Verification items for the finished model (mm, model axes). Face numbers are marked on the shaded views. Coordinates: 2 decimals unless noted, no trailing zeros. Write each loop counter-clockwise with the first axis right and the second up, starting at its lowest first coordinate (ties: lowest second). Pieces come first, ordered by that corner, then holes. Notation, with made-up numbers: (-7.5, 5.5) - (37.5, 5.5) arc R20 cw to (37.5, 10.5) - close; hole circle Ø2 at (-14.75, 86.5). An arc over 180 degrees is marked (long way). Use one line per item in the form item = value. Start each with the question number.
(1) Sectioned sample at C-C (x = 6.5). Record the cut outline in (y, z), and give its area (3 significant figures).
(2) Sectioned sample at B-B (y = -48). Record the cut outline in (x, z), and give its area (3 significant figures).
(3) Gauge pin test, flat ends, axial feed: pin 1 Ø4 at (y, z) = (24, -41.57) entering from -X; pin 2 Ø3 at (x, y) = (1.5, 21) entering from -Z; pin 3 Ø3 at (x, z) = (6, -33) entering from +Y; pin 4 Ø3 at (x, z) = (3, -19) entering from -Y. Record the tip position at first contact, or that the pin passes through.
(4) Sectioned sample at A-A (z = 0). Count the separate pieces of the cut face and the enclosed holes in it, and give its area (3 significant figures).
(5) Material ranges on line 1 (Y direction, x = 1.1, z = 0); line 2 (Y direction, x = 6.85, z = 0); line 3 (Z direction, x = 7, y = -15.5), recorded low to high. Write a range as [from, to].
(6) Mould release check, pull along Z, two halves, no side actions. Record for the marked faces 1, 2 and 3: released by +Z, released by -Z, zero draft, split by the parting line, or undercut.
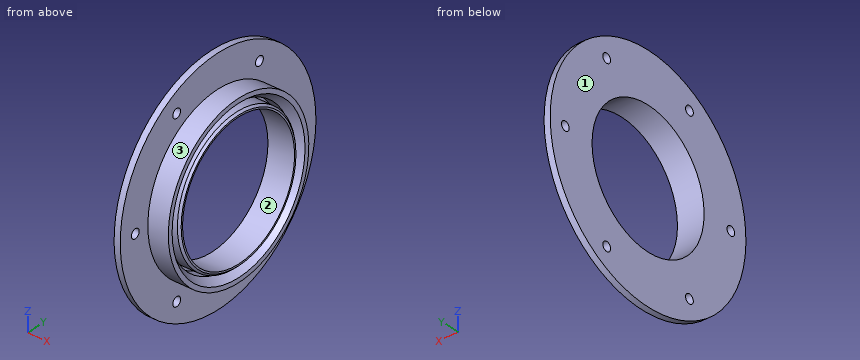
from build123d import *

# Parameters (mm, degrees)
CHAMFER1_SIZE      = 4
CHAMFER1_SIZE2     = 2.800830153
CHAMFER2_SIZE      = 1
SKETCH2_R          = 2.25
CUT_EXTRUDE1_DEPTH = 10
CIRPATTERN1_COUNT  = 6


with BuildPart() as part:
    # Sketch1 → Revolve1 (revolve)
    with BuildSketch(Plane.XY, mode=Mode.PRIVATE) as revolve1_sk:
        Polygon((0, 32.5), (13, 32.5), (13, 34.3), (3, 34.3), (3, 35.75), (13, 35.75), (13, 40.75), (3, 40.75), (3, 56.75), (0, 56.75), align=None)
    revolve(revolve1_sk.sketch.rotate(Axis((0, 0, 0), (1, 0, 0)), 90), axis=Axis((0, 0, 0), (1, 0, 0)))

    # Chamfer1
    chamfer1_edges = [part.edges().sort_by_distance(p)[0] for p in [
        (13, 0, -35.75),
    ]]
    chamfer1_side = [part.faces().sort_by_distance(p)[0] for p in [
        (8, 0, -35.75),
    ]]
    chamfer(chamfer1_edges, length=CHAMFER1_SIZE, length2=CHAMFER1_SIZE2, reference=chamfer1_side[0])

    # Chamfer2
    chamfer2_edges = [part.edges().sort_by_distance(p)[0] for p in [
        (13, 0, -34.3),
    ]]
    chamfer(chamfer2_edges, length=CHAMFER2_SIZE)

    # Sketch2 → Cut-Extrude1 (cut)
    with BuildSketch(Plane(origin=(3, 0, 0), x_dir=(0, 0, -1), z_dir=(1, 0, 0))):
        with Locations((0, 48)):
            Circle(SKETCH2_R)
    cut_extrude1 = extrude(amount=-CUT_EXTRUDE1_DEPTH, mode=Mode.SUBTRACT)

    # CirPattern1: Cut-Extrude1 ×6 about axis
    cirpattern1_axis = Axis((0, 0, 0), (1, 0, 0))
    for i in range(1, CIRPATTERN1_COUNT):
        add(cut_extrude1.rotate(cirpattern1_axis, i * 360 / CIRPATTERN1_COUNT), mode=Mode.SUBTRACT)


solid = part.part
Answers below:
q1.outline = circle Ø81.5 at (0, 0); circle Ø68.6 at (0, 0); hole circle Ø71.5 at (0, 0); hole circle Ø65 at (0, 0)
q1.area = 1,580 mm2
q2.outline = (0, -30.27) - (3, -30.27) - (3, -2.25) - (0, -2.25) - close; (0, 2.25) - (3, 2.25) - (3, 30.27) - (0, 30.27) - close
q2.area = 168 mm2
q3.pin_1 = through
q3.pin_2 = -53.29
q3.pin_3 = 25.85
q3.pin_4 = -53.98
q4.separate_pieces = 4
q4.enclosed_holes = 0
q4.area = 242 mm2
q5.line_1 = [-56.75, -50.25], [-45.75, -32.5], [32.5, 45.75], [50.25, 56.75]
q5.line_2 = [-40.75, -35.75], [-34.3, -32.5], [32.5, 34.3], [35.75, 40.75]
q5.line_3 = [-37.69, -32.22], [-30.6, -28.57], [28.57, 30.6], [32.22, 37.69]
q6.face_1 = zero draft
q6.face_2 = undercut
q6.face_3 = split by the parting line
